```python
from build123d import *

# Parameters (mm, degrees)
SKETCH_2_W                  = 49
SKETCH_2_H                  = 23
SHELL_1_T                   = -3
SKETCH_11_W                 = 54
SKETCH_11_H                 = 23
SKETCH_11_W_2               = 43
SKETCH_11_H_2               = 12
EXTRUDE_1_DEPTH             = 22
SKETCH_12_W                 = 23.011901601
SKETCH_12_H                 = 37
CUT_EXTRUDE_9_DEPTH         = 767.019092451
HOLE_WIZARD_4_2_4_2_1_D     = 4.2
SKETCH_15_W                 = 54
SKETCH_15_H                 = 23
SKETCH_15_W_2               = 43
SKETCH_15_H_2               = 12
EXTRUDE_2_DEPTH             = 22
SKETCH_16_W                 = 45.795478168
SKETCH_16_H                 = 37
CUT_EXTRUDE_10_DEPTH        = 49
HOLE_WIZARD_4_2_4_2_2_D     = 4.2
HOLE_WIZARD_4_2_4_2_2_DEPTH = 50
HOLE_WIZARD_4_2_4_2_2_TIP   = 1.2618073


with BuildPart() as part:
    # 扫描1: sweep along a path in 草图1
    with BuildLine(Plane.XY) as sweep_1_path:
        Line((0, 0), (-700, 0))
        ThreePointArc((-700, 0), (-748, 48), (-700, 96))
        Line((-700, 96), (-580, 96))
    # 草图2 → 扫描1 (sweep)
    with BuildSketch(Plane(origin=(0, 0, 0), x_dir=(0, 0, -1), z_dir=(1, 0, 0))):
        Rectangle(SKETCH_2_W, SKETCH_2_H)
    sweep(path=sweep_1_path.line)

    # 抽壳1
    shell_1_openings = [part.faces().sort_by_distance(p)[0] for p in [
        (-580, 96, 0),
        (0, 0, 0),
    ]]
    offset(amount=SHELL_1_T, openings=shell_1_openings, kind=Kind.INTERSECTION)

    # 草图11 → 凸台-拉伸1 (add)
    with BuildSketch(Plane(origin=(0, 0, 0), x_dir=(0, 0, -1), z_dir=(1, 0, 0))):
        Rectangle(SKETCH_11_W, SKETCH_11_H)
        Rectangle(SKETCH_11_W_2, SKETCH_11_H_2, mode=Mode.SUBTRACT)
    extrude(amount=EXTRUDE_1_DEPTH)

    # 草图12 → 切除-拉伸9 (cut, through all)
    with BuildSketch(Plane(origin=(0, 11.5, 0), x_dir=(1, 0, 0), z_dir=(0, 1, 0))):
        with Locations((11.505950801, 0)):
            Rectangle(SKETCH_12_W, SKETCH_12_H)
    extrude(amount=-CUT_EXTRUDE_9_DEPTH, mode=Mode.SUBTRACT)

    # Ø4.2 (4.2) 直径孔1 (through all)
    with Locations(Plane(origin=(0, 11.5, 0), x_dir=(1, 0, 0), z_dir=(0, 1, 0))):
        with Locations((12, 23.5), (12, -23.5)):
            Hole(HOLE_WIZARD_4_2_4_2_1_D / 2)

    # 草图15 → 凸台-拉伸2 (add)
    with BuildSketch(Plane(origin=(-580, 0, 0), x_dir=(0, 0, -1), z_dir=(1, 0, 0))):
        with Locations((0, 96)):
            Rectangle(SKETCH_15_W, SKETCH_15_H)
        with Locations((0, 96)):
            Rectangle(SKETCH_15_W_2, SKETCH_15_H_2, mode=Mode.SUBTRACT)
    extrude(amount=EXTRUDE_2_DEPTH)

    # 草图16 → 切除-拉伸10 (cut)
    with BuildSketch(Plane(origin=(0, 107.5, 0), x_dir=(1, 0, 0), z_dir=(0, 1, 0))):
        with Locations((-557.102260916, 0)):
            Rectangle(SKETCH_16_W, SKETCH_16_H)
    extrude(amount=-CUT_EXTRUDE_10_DEPTH, mode=Mode.SUBTRACT)

    # Ø4.2 (4.2) 直径孔2
    with Locations(Plane(origin=(0, 107.5, 0), x_dir=(1, 0, 0), z_dir=(0, 1, 0))):
        with Locations((-568, 23.5), (-568, -23.5)):
            Hole(HOLE_WIZARD_4_2_4_2_2_D / 2, depth=HOLE_WIZARD_4_2_4_2_2_DEPTH)
            with Locations((0, 0, -(HOLE_WIZARD_4_2_4_2_2_DEPTH + HOLE_WIZARD_4_2_4_2_2_TIP / 2))):  # 118° drill point
                Cone(0, HOLE_WIZARD_4_2_4_2_2_D / 2, HOLE_WIZARD_4_2_4_2_2_TIP, mode=Mode.SUBTRACT)


solid = part.part
```
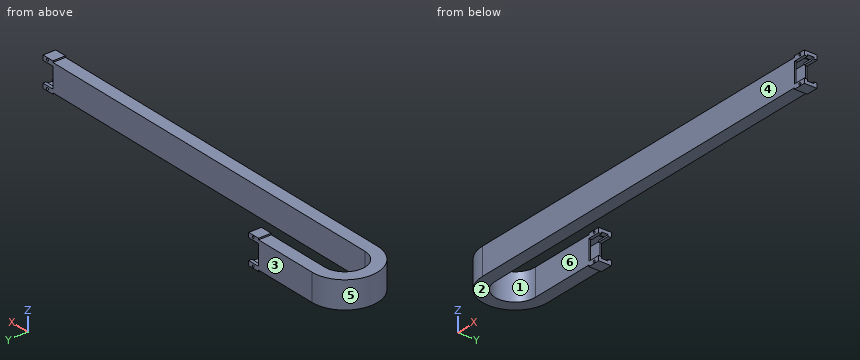
Geometry: final body of the model. Coordinates: model frame, mm. Face numbers are marked on the shaded views. A direction names the side the tool comes from. Coordinates: 2 decimals unless noted, no trailing zeros. Order: outer loops, then holes, each group sorted by start corner. A loop starts at its lowest first (then second) coordinate and runs counter-clockwise, first axis right, second up. Notation, with made-up numbers: (-38.75, -22.75) -> (-3.75, -22.75) arc R26 cw to (-3.75, 10.25) -> close; hole circle Ø11 at (-37.75, 24). An arc over 180 degrees is marked (long way). Answer in a Markdown table with one row per item.
Item 1: Draft query along Y for the marked faces 1, 2, 3 and 4. Return one class per face: released by +Y, released by -Y, zero draft, split by the parting line, or undercut.
Return value:
| item | result |
|---|---|
| face 1 | undercut |
| face 2 | zero draft |
| face 3 | released by +Y |
| face 4 | released by -Y |
Item 2: Ray query, L1, parallel to Y at x = -597.5, z = -20.5; L2, parallel to Y at x = -504.5, z = 12; L3, parallel to Z at x = 12, y = 7. Return the intervals inside material, ascending.
Return value:
| item | result |
|---|---|
| L1 | y = -11.5 to -8.5, 8.5 to 11.5, 84.5 to 87.5, 104.5 to 107.5 |
| L2 | y = -11.5 to -8.5, 8.5 to 11.5 |
| L3 | z = -27 to -25.6, -21.4 to -18.5, 18.5 to 21.4, 25.6 to 27 |
Item 3: Section C-C on z = 3.5. Output: boundary loops of the cut face in (x, y).
Return value:
| item | result |
|---|---|
| outline | (-700, -11.5) -> (0, -11.5) -> (0, -8.5) -> (-700, -8.5) arc R56.5 cw to (-700, 104.5) -> (-580, 104.5) -> (-580, 107.5) -> (-700, 107.5) arc R59.5 ccw to start; (-700, 8.5) -> (0, 8.5) -> (0, 11.5) -> (-700, 11.5) arc R36.5 cw to (-700, 84.5) -> (-580, 84.5) -> (-580, 87.5) -> (-700, 87.5) arc R39.5 ccw to start |
Item 4: Section D-D on y = 48. Output: boundary loops of the cut face in (x, z).
Return value:
| item | result |
|---|---|
| outline | (-759.5, -24.5) -> (-736.5, -24.5) -> (-736.5, 24.5) -> (-759.5, 24.5) -> close; hole (-756.5, -21.5) -> (-739.5, -21.5) -> (-739.5, 21.5) -> (-756.5, 21.5) -> close |
Item 5: Access query for the marked faces 5 and 6. Directions: +Z, -Z, +X, -X, +Y, -Y. A direction counts if a zero-diameter tool reaches every point of the face in a straight line with its end or side. Return the directions, or none.
Return value:
| item | result |
|---|---|
| face 5 | +Z, -Z, -X |
| face 6 | +Z, -Z, +X |
Item 6: Contact query for flat-ended pins moving along their axis: P1, Ø2, axis at y = 93, z = -21, coming from the +X side; P2, Ø3.5, axis at x = 15, z = -20, coming from the +Y side; P3, Ø12, axis at x = -89.5, y = 16, coming from the +Z side; P4, Ø5, axis at x = 12, z = 23.5, coming from the -Y side. Output: stop coordinate, or through.
Return value:
| item | result |
|---|---|
| P1 | stops at x = -558 |
| P2 | stops at y = 11.5 |
| P3 | stops at z = 24.5 |
| P4 | stops at y = -11.5 |
Item 7: Section B-B on x = -380.5. Output: boundary loops of the cut face in (y, z), plus the area to 3 significant figures.
Return value:
| item | result |
|---|---|
| outline | (-11.5, -24.5) -> (11.5, -24.5) -> (11.5, 24.5) -> (-11.5, 24.5) -> close; hole (-8.5, -21.5) -> (8.5, -21.5) -> (8.5, 21.5) -> (-8.5, 21.5) -> close |
| area | 396 mm² |
Item 8: Section A-A on x = -674. Output: boundary loops of the cut face in (y, z).
Return value:
| item | result |
|---|---|
| outline | (-11.5, -24.5) -> (11.5, -24.5) -> (11.5, 24.5) -> (-11.5, 24.5) -> close; (84.5, -24.5) -> (107.5, -24.5) -> (107.5, 24.5) -> (84.5, 24.5) -> close; hole (-8.5, -21.5) -> (8.5, -21.5) -> (8.5, 21.5) -> (-8.5, 21.5) -> close; hole (87.5, -21.5) -> (104.5, -21.5) -> (104.5, 21.5) -> (87.5, 21.5) -> close |
